Part print with two shaded views. Sizes in mm from the minimum x, y, z corner. Give positions to 0.01 mm unless a question says otherwise; leave off trailing zeros. Write each loop counter-clockwise with the first axis right and the second up, starting at its lowest first coordinate (ties: lowest second). Pieces come first, ordered by that corner, then holes. Notation, with made-up numbers: M -4,-29.75 L 1,-29.75 A17 cw 1,-0.75 Z; hole C 41.5,-39.75 d10. An arc over 180 degrees is marked long. Return JSON: item names as keys, results as strings. Group by question number.
Q1. Band-saw the part on A-A, the plane y = 75. Give the cut face in (x, z).
Q2. Flat gauge pins, fed straight in: pin 1 Ø6 at (y, z) = (52.5, 13) entering from -X; pin 2 Ø3 at (x, z) = (82, 7) entering from -Y; pin 3 Ø3 at (y, z) = (42.5, 7.5) entering from -X. Where does each tip first touch, or does it go through?
Q3. Band-saw the part on D-D, the plane y = 108.75. Give the cut face in (x, z).
Q4. Band-saw the part on B-B, the plane z = 4.75. Count the separate pieces of the cut face and the enclosed holes in it, then the cut area to 3 significant figures.
Q5. Band-saw the part on C-C, the plane x = 53. Give the cut face in (y, z), then the cut area to 3 significant figures.
Q6. Wall check: probe 1 along Y at (x, z) = (75, 9) (1 decimal); probe 2 along Z at (x, y) = (87, 13.5); probe 3 along Y at (x, z) = (108.5, 15.75). Give the ranges that are in metal, low to high.
Q7. Pull direction X, two halves, no side cores. Call the marked faces 1, 2 and 3: +X half, -X half, draft (parallel to the pull), parting line (faces both ways), or undercut.
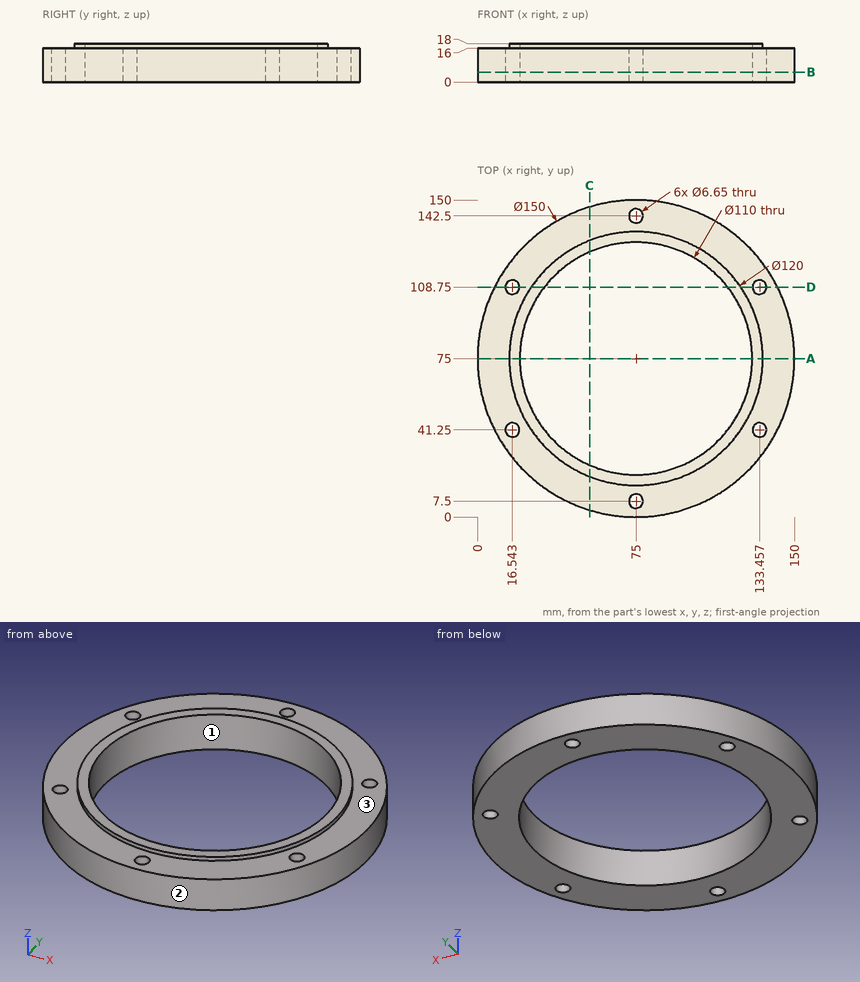
From the geometry:
{
 "1": {"outline": "M 0,0 L 20,0 L 20,18 L 15,18 L 15,16 L 0,16 Z; M 130,0 L 150,0 L 150,16 L 135,16 L 135,18 L 130,18 Z"},
 "2": {"pin 1": "stops at x = 2.58", "pin 2": "stops at y = 0.2", "pin 3": "stops at x = 6.71"},
 "3": {"outline": "M 8.02,0 L 13.22,0 L 13.22,16 L 8.02,16 Z; M 19.87,0 L 31.57,0 L 31.57,18 L 25.39,18 L 25.39,16 L 19.87,16 Z; M 118.43,0 L 130.13,0 L 130.13,16 L 124.61,16 L 124.61,18 L 118.43,18 Z; M 136.78,0 L 141.98,0 L 141.98,16 L 136.78,16 Z"},
 "4": {"separate pieces": "1", "enclosed holes": "7", "area": "7,960 mm^2"},
 "5": {"outline": "M 3.3,0 L 24.59,0 L 24.59,18 L 19.18,18 L 19.18,16 L 3.3,16 Z; M 125.41,0 L 146.7,0 L 146.7,16 L 130.82,16 L 130.82,18 L 125.41,18 Z", "area": "703 mm^2"},
 "6": {"probe 1": "y = 0 to 4.2, 10.8 to 20, 130 to 139.2, 145.8 to 150", "probe 2": "z = 0 to 16", "probe 3": "y = 7.9 to 31.38, 118.62 to 142.1"},
 "7": {"face 1": "undercut", "face 2": "parting line", "face 3": "draft"}
}
